Drawing for the job (mm, zero at the part's lowest x, y, z). Coordinates: 2 decimals unless noted, no trailing zeros. Loops run counter-clockwise (first coordinate to the right, second up) from the corner with the lowest first, then second, coordinate; pieces in that order, holes last. Notation, with made-up numbers: (-33.5, -24.75) -> (2.5, -24.75) arc R5 cw to (2.5, -17.75) -> close; hole circle Ø5 at (51, -4). An arc over 180 degrees is marked (long way). Write each question's results on one line, items separated by ' | '.
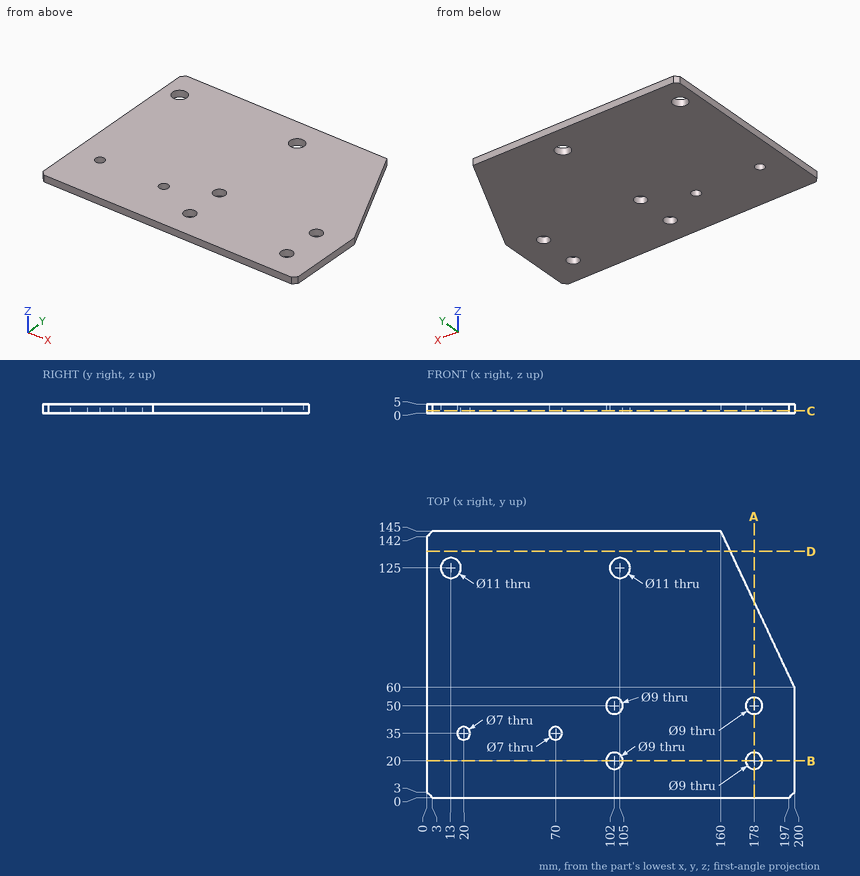
1) Slice it at B-B (y = 20). Write the cut outline in (x, z).
Outcome:
outline: (0, 0) -> (97.5, 0) -> (97.5, 5) -> (0, 5) -> close; (106.5, 0) -> (173.5, 0) -> (173.5, 5) -> (106.5, 5) -> close; (182.5, 0) -> (200, 0) -> (200, 5) -> (182.5, 5) -> close
2) Slice it at C-C (z = 1.25). Count the separate pieces of the cut face and the enclosed holes in it, then the cut area to 3 significant figures.
Outcome:
separate pieces: 1 | enclosed holes: 8 | area: 26,800 mm^2
3) Slice it at D-D (y = 134). Write the cut outline in (x, z), then the cut area to 3 significant figures.
Outcome:
outline: (0, 0) -> (165.18, 0) -> (165.18, 5) -> (0, 5) -> close | area: 826 mm^2
4) Drill centre lines: L1, parallel to X at y = 20, z = 1.2; L2, parallel to Y at x = 70, z = 3.75; L3, parallel to Y at x = 103, z = 1.4. Where is each one in solid material? Low to high. Write a range as from..to.
Outcome:
L1: x = 0..97.5, 106.5..173.5, 182.5..200 | L2: y = 0..31.5, 38.5..145 | L3: y = 0..15.61, 24.39..45.61, 54.39..119.88, 130.12..145
5) Slice it at A-A (x = 178). Write the cut outline in (y, z).
Outcome:
outline: (0, 0) -> (15.5, 0) -> (15.5, 5) -> (0, 5) -> close; (24.5, 0) -> (45.5, 0) -> (45.5, 5) -> (24.5, 5) -> close; (54.5, 0) -> (106.75, 0) -> (106.75, 5) -> (54.5, 5) -> close
